Verification items for the finished model (mm, model axes). Face numbers are marked on the shaded views. A direction names the side the tool comes from. Give positions to 0.01 mm unless a question says otherwise; leave off trailing zeros. Order: outer loops, then holes, each group sorted by start corner. A loop starts at its lowest first (then second) coordinate and runs counter-clockwise, first axis right, second up. Notation, with made-up numbers: (44.5, 34) -> (54.5, 34) arc R36 ccw to (54.5, 71) -> close; hole circle Ø2 at (75, 32.5). An arc over 180 degrees is marked (long way). Return JSON: item names as keys, results as strings. Group by question number.
(1) Cross-section at A-A on y = 5. Enter the section's corners in (x, z).
(2) Thickness scan on line 1 along Y through (x, z) = (-36, 64); line 2 along X through (y, z) = (-5.5, 63); line 3 along Y through (x, z) = (48.5, 41). Record the ranges inside material, lowest first.
(3) Depth check by flat-ended pin: pin 1 Ø5 at (x, z) = (47.5, 38) entering from -Y. Enter the tip coordinate at first touch or a pass-through.
(4) Tool access check on the marked faces 1 and 2. Record the directions out of +Z, -Z, +X, -X, +Y, -Y that give a thin tool (end or side, any length) a straight path to the whole face; none if there is none.
(5) Release check for a two-part mould opening along Y. For the marked faces 3, 4, 5 and 6 record: pulls with the +Y half, pulls with the -Y half, needs draft (parallel to the pull), parting line crosses it, or undercut.
(6) Cross-section at C-C on z = 97.5. Enter the section's corners in (x, y), then the cut area to 3 significant figures.
(7) Cross-section at B-B on x = 35. Enter the section's corners in (y, z).
from build123d import *

# Parameters (mm, degrees)
SKETCH_1_W      = 120
SKETCH_1_H      = 80
SKETCH_1_W_2    = 102
SKETCH_1_H_2    = 62
EXTRUDE_1_DEPTH = 118
FILLET_1_R      = 15
FILLET_2_R      = 6


with BuildPart() as part:
    # 草图1 → 凸台-拉伸1 (new body)
    with BuildSketch(Plane.XY):
        Rectangle(SKETCH_1_W, SKETCH_1_H)
        Rectangle(SKETCH_1_W_2, SKETCH_1_H_2, mode=Mode.SUBTRACT)
    extrude(amount=EXTRUDE_1_DEPTH)

    # 圆角1
    fillet_1_edges = [part.edges().sort_by_distance(p)[0] for p in [
        (-60, 40, 59),
        (60, 40, 59),
        (60, -40, 59),
        (-60, -40, 59),
    ]]
    fillet(fillet_1_edges, radius=FILLET_1_R)

    # 圆角2
    fillet_2_edges = [part.edges().sort_by_distance(p)[0] for p in [
        (-51, 31, 59),
        (-51, -31, 59),
        (51, -31, 59),
        (51, 31, 59),
    ]]
    fillet(fillet_2_edges, radius=FILLET_2_R)


solid = part.part
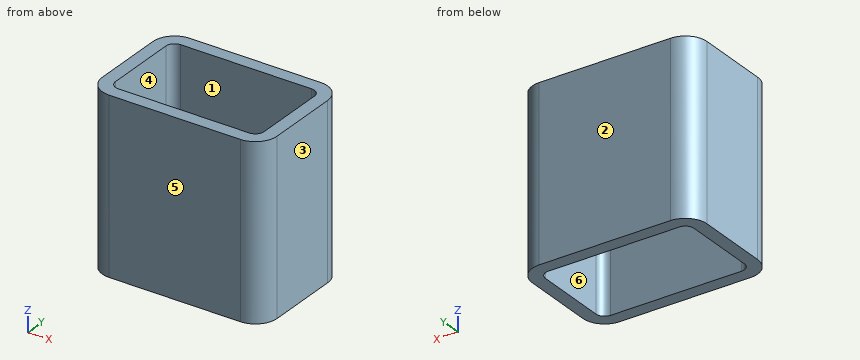
Verdict:
{
 "1": {"outline": "(-60, 0) -> (-51, 0) -> (-51, 118) -> (-60, 118) -> close; (51, 0) -> (60, 0) -> (60, 118) -> (51, 118) -> close"},
 "2": {"line 1": "-40 to -31, 31 to 40", "line 2": "-60 to -51, 51 to 60", "line 3": "-39.59 to -29.87, 29.87 to 39.59"},
 "3": {"pin 1": "y = -40"},
 "4": {"face 1": "+Z, -Z", "face 2": "+Z, -Z, +X, -X, +Y"},
 "5": {"face 3": "needs draft", "face 4": "undercut", "face 5": "pulls with the -Y half", "face 6": "undercut"},
 "6": {"outline": "(-60, -25) arc R15 ccw to (-45, -40) -> (45, -40) arc R15 ccw to (60, -25) -> (60, 25) arc R15 ccw to (45, 40) -> (-45, 40) arc R15 ccw to (-60, 25) -> close; hole (-51, -25) arc R6 ccw to (-45, -31) -> (45, -31) arc R6 ccw to (51, -25) -> (51, 25) arc R6 ccw to (45, 31) -> (-45, 31) arc R6 ccw to (-51, 25) -> close", "area": "3,110 mm²"},
 "7": {"outline": "(-40, 0) -> (-31, 0) -> (-31, 118) -> (-40, 118) -> close; (31, 0) -> (40, 0) -> (40, 118) -> (31, 118) -> close"}
}
